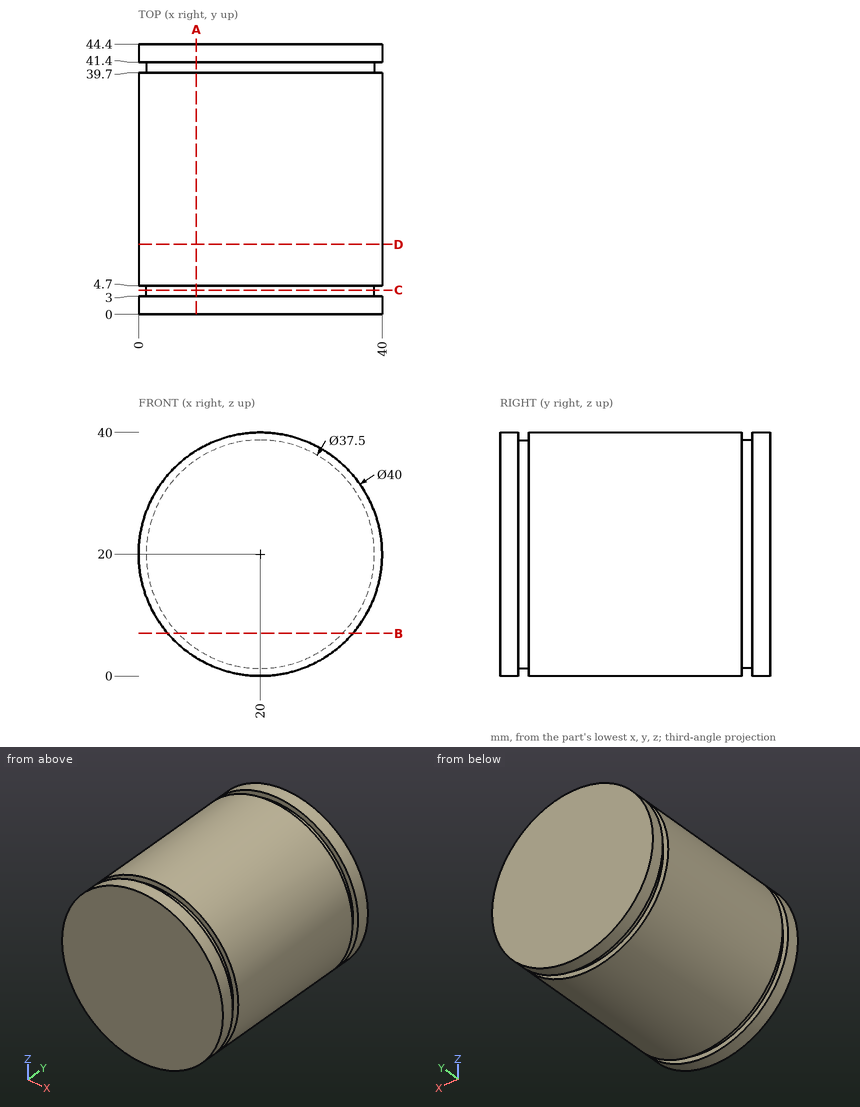
Print and shaded views of the part. All mm, measured from the part's lowest x, y and z. Coordinates: 2 decimals unless noted, no trailing zeros. Order: outer loops, then holes, each group sorted by start corner. A loop starts at its lowest first (then second) coordinate and runs counter-clockwise, first axis right, second up. Notation, with made-up numbers: (88, 48) -> (96, 48) arc R21 ccw to (96, 70) -> close; hole circle Ø3 at (8, 23). An arc over 180 degrees is marked (long way). Answer as a JSON object with one key per item and string values. Group by question number.
1) Flat gauge pins, fed straight in: pin 1 (1 mm diameter, centred on x = 11.5, y = 15.5, fed in from +Z); pin 2 (3 mm diameter, centred on y = 19.5, z = 11.5, fed in from +X) (3 decimals); pin 3 (3 mm diameter, centred on y = 15, z = 5.5, fed in from +X). Where does each tip first touch, or does it go through?
2) Drill centre lines: L1, parallel to Y at x = 9, z = 3.5; L2, parallel to X at y = 28.5, z = 5.5; L3, parallel to X at y = 6, z = 35.5. Where is each one in solid material? Low to high.
3) Cut at A-A, the plane x = 9.5. Write the cut outline in (y, z).
4) Cut at D-D, the plane y = 11.5. Write the cut outline in (x, z), then the cut area to 3 significant figures.
5) Cut at B-B, the plane z = 7. Write the cut outline in (x, y).
6) Cut at C-C, the plane y = 4. Write the cut outline in (x, z), then the cut area to 3 significant figures.
Check values:
{
 "1": {"pin 1": "stops at z = 38.33", "pin 2": "stops at x = 38.735", "pin 3": "stops at x = 35.2"},
 "2": {"L1": "y = 0 to 3, 4.7 to 39.7, 41.4 to 44.4", "L2": "x = 6.23 to 33.77", "L3": "x = 7.36 to 32.64"},
 "3": {"outline": "(0, 2.98) -> (3, 2.98) -> (3, 4.47) -> (4.7, 4.47) -> (4.7, 2.98) -> (39.7, 2.98) -> (39.7, 4.47) -> (41.4, 4.47) -> (41.4, 2.98) -> (44.4, 2.98) -> (44.4, 37.02) -> (41.4, 37.02) -> (41.4, 35.53) -> (39.7, 35.53) -> (39.7, 37.02) -> (4.7, 37.02) -> (4.7, 35.53) -> (3, 35.53) -> (3, 37.02) -> (0, 37.02) -> close"},
 "4": {"outline": "circle Ø40 at (20, 20)", "area": "1,260 mm²"},
 "5": {"outline": "(4.8, 0) -> (35.2, 0) -> (35.2, 3) -> (33.51, 3) -> (33.51, 4.7) -> (35.2, 4.7) -> (35.2, 39.7) -> (33.51, 39.7) -> (33.51, 41.4) -> (35.2, 41.4) -> (35.2, 44.4) -> (4.8, 44.4) -> (4.8, 41.4) -> (6.49, 41.4) -> (6.49, 39.7) -> (4.8, 39.7) -> (4.8, 4.7) -> (6.49, 4.7) -> (6.49, 3) -> (4.8, 3) -> close"},
 "6": {"outline": "circle Ø37.5 at (20, 20)", "area": "1,100 mm²"}
}
